Can you work these out from the model? Positions are in its coordinate system, mm. Give positions to 0.01 mm unless a question says otherwise; leave off trailing zeros. Loops run counter-clockwise (first coordinate to the right, second up) from the corner with the lowest first, then second, coordinate; pieces in that order, holes last. Notation, with made-up numbers: M 80,43 L 128,43 A22 ccw 128,54 Z; hole C 1,-27.75 d7. An arc over 180 degrees is marked long. Use CSV: the item, a comma, the result in double quotes.
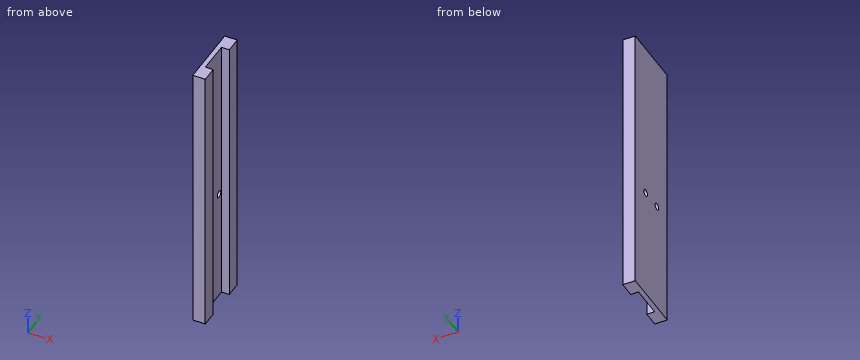
from build123d import *

# Parameters (mm, degrees)
BOSS_EXTRUDE1_DEPTH  = 900
F_1_8_TAPPED_HOLE1_D = 22.225


with BuildPart() as part:
    # Sketch1 → Boss-Extrude1 (new body)
    with BuildSketch(Plane.XY):
        Polygon((0, 0), (0, 200), (40, 200), (40, 150.25), (15, 150.25), (15, 49.75), (40, 49.75), (40, 0), align=None)
    extrude(amount=BOSS_EXTRUDE1_DEPTH)

    # 1-8 Tapped Hole1 (through all)
    with Locations(Plane(origin=(15, 135, 370), x_dir=(0, 1, 0), z_dir=(1, 0, 0))):
        with Locations((0, 0), (-70, 0)):
            Hole(F_1_8_TAPPED_HOLE1_D / 2)


solid = part.part
Q1. Please list where these lines run through material, in increasing order: L1, parallel to Y at x = 30.5, z = 162; L2, parallel to Z at x = 5.5, y = 65; L3, parallel to X at y = 77, z = 83.5. Write a range as from..to.
Model answer:
L1,"0..49.75, 150.25..200"
L2,"0..358.89, 381.11..900"
L3,"0..15"
Q2. I want a section at A-A, the plane y = 135. Please give me the cut outline in (x, z), then the cut area to 3 significant figures.
Model answer:
outline,"M 0,0 L 15,0 L 15,358.89 L 0,358.89 Z; M 0,381.11 L 15,381.11 L 15,900 L 0,900 Z"
area,"13,200 mm2"
Q3. I want a section at B-B, the plane z = 370. Please give me the cut outline in (x, y), then the cut area to 3 significant figures.
Model answer:
outline,"M 0,0 L 40,0 L 40,49.75 L 15,49.75 L 15,53.89 L 0,53.89 Z; M 0,76.11 L 15,76.11 L 15,123.89 L 0,123.89 Z; M 0,146.11 L 15,146.11 L 15,150.25 L 40,150.25 L 40,200 L 0,200 Z"
area,"4,820 mm2"
Q4. I'm going to push a flat-ended pin straight in: P1, Ø13.5, axis at y = 65, z = 370, coming from the -X side. Where does the tip first touch, or does it pass through?
Model answer:
P1,"through"
